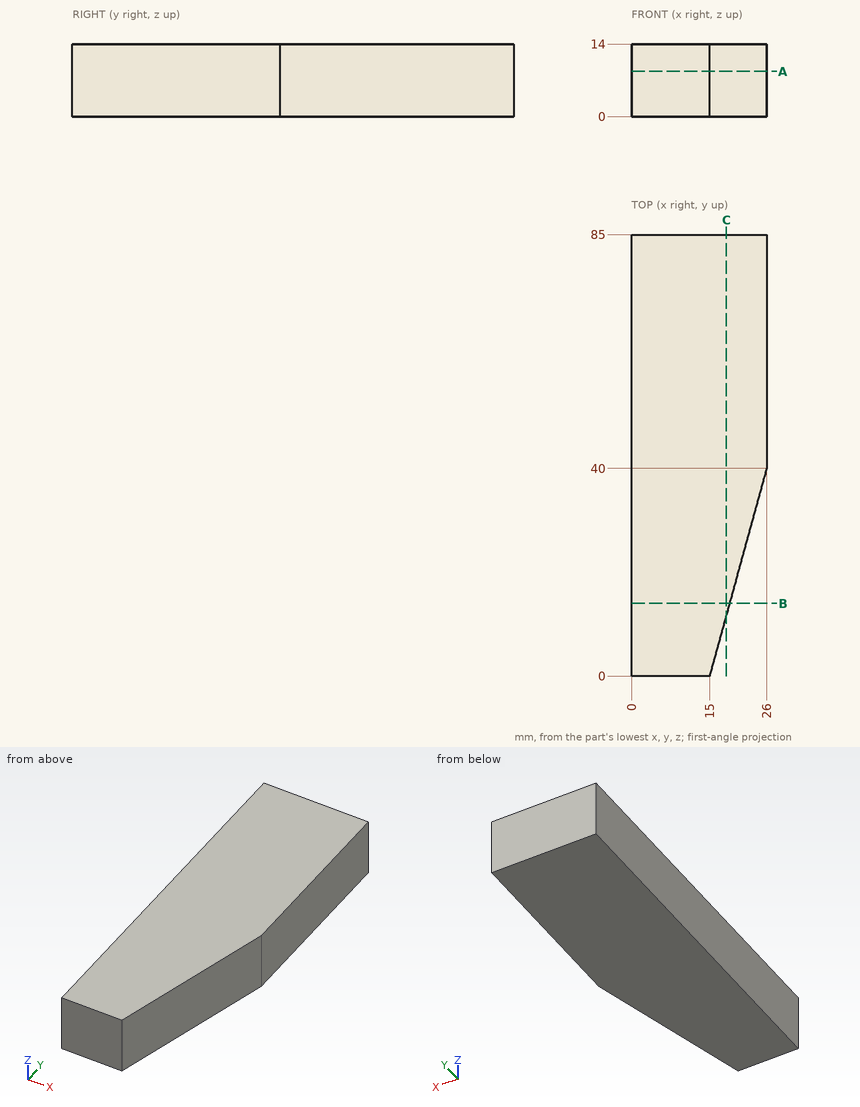
Check sheet for the drawn part. Datum: minimum x, y, z corner. Units: mm. Round coordinates to 2 decimals unless told otherwise and drop trailing zeros. Loops run counter-clockwise (first coordinate to the right, second up) from the corner with the lowest first, then second, coordinate; pieces in that order, holes last. Notation, with made-up numbers: M 20.5,69 L 73.5,69 A13 ccw 73.5,94 Z; hole C 61.25,85 d9. An arc over 180 degrees is marked long. One line per question, with ' | ' between items. Start each with the question number.
Item 1: Scan lines: probe 1 along X at (y, z) = (26.5, 12.75); probe 2 along X at (y, z) = (25, 5.25) (3 decimals). Record each from-to range of solid material in increasing order.
Item 2: Section check C-C (x = 18.25). Record the boundary of the cut face in (y, z), and give its area (3 significant figures).
Item 3: Gauge pin test, flat end, axial feed: pin 1 Ø4 at (y, z) = (19, 5) entering from +X (3 decimals). Record the tip position at first contact, or that the pin passes through.
Item 4: Section check B-B (y = 14). Record the boundary of the cut face in (x, z).
Item 5: Section check A-A (z = 8.75). Record the boundary of the cut face in (x, y).
Worked out:
1) probe 1: 0 to 22.29 | probe 2: 0 to 21.875
2) outline: M 11.82,0 L 85,0 L 85,14 L 11.82,14 Z | area: 1,020 mm^2
3) pin 1: x = 20.775
4) outline: M 0,0 L 18.85,0 L 18.85,14 L 0,14 Z
5) outline: M 0,0 L 15,0 L 26,40 L 26,85 L 0,85 Z
